from build123d import *

# Parameters (mm, degrees)
SKETCH_1_W             = 15
SKETCH_1_H             = 26
EXTRUDE_1_DEPTH        = 40
HOLE_WIZARD_M6_1_D     = 5
HOLE_WIZARD_M6_1_DEPTH = 15
HOLE_WIZARD_M6_1_TIP   = 1.502151548
HOLE_WIZARD_M6_2_D     = 5
HOLE_WIZARD_M6_2_DEPTH = 15
HOLE_WIZARD_M6_2_TIP   = 1.502151548
CHAMFER_2_SIZE         = 10


with BuildPart() as part:
    # 草图1 → 凸台-拉伸1 (new body)
    with BuildSketch(Plane.XY):
        Rectangle(SKETCH_1_W, SKETCH_1_H)
    extrude(amount=EXTRUDE_1_DEPTH)

    # M6 螺纹孔1
    with Locations(Plane(origin=(0, 13, 0), x_dir=(1, 0, 0), z_dir=(0, 1, 0))):
        with Locations((0, -12), (0, -28)):
            Hole(HOLE_WIZARD_M6_1_D / 2, depth=HOLE_WIZARD_M6_1_DEPTH)
            with Locations((0, 0, -(HOLE_WIZARD_M6_1_DEPTH + HOLE_WIZARD_M6_1_TIP / 2))):  # 118° drill point
                Cone(0, HOLE_WIZARD_M6_1_D / 2, HOLE_WIZARD_M6_1_TIP, mode=Mode.SUBTRACT)

    # M6 螺纹孔2
    with Locations(Plane(origin=(0, 0, 0), x_dir=(-1, 0, 0), z_dir=(0, 0, -1))):
        with Locations((0, 0)):
            Hole(HOLE_WIZARD_M6_2_D / 2, depth=HOLE_WIZARD_M6_2_DEPTH)
            with Locations((0, 0, -(HOLE_WIZARD_M6_2_DEPTH + HOLE_WIZARD_M6_2_TIP / 2))):  # 118° drill point
                Cone(0, HOLE_WIZARD_M6_2_D / 2, HOLE_WIZARD_M6_2_TIP, mode=Mode.SUBTRACT)

    # 倒角2
    chamfer_2_edges = [part.edges().sort_by_distance(p)[0] for p in [
        (0, -13, 40),
    ]]
    chamfer(chamfer_2_edges, length=CHAMFER_2_SIZE)


solid = part.part
The model under review builds one solid part; all positions refer to its coordinate system, in mm. A direction names the side the tool comes from. Round coordinates to 2 decimals unless told otherwise and drop trailing zeros. Loops run counter-clockwise (first coordinate to the right, second up) from the corner with the lowest first, then second, coordinate; pieces in that order, holes last. Notation, with made-up numbers: M 13.25,52 L 36.25,52 A32 ccw 36.25,87 Z; hole C 82.25,-37 d4. An arc over 180 degrees is marked long. Answer as a JSON object with one key per item and string values.
Item 1: We need section A-A, the plane y = 7. State the section outline as (x, z) points, and give its area (3 significant figures).
Check sheet entries:
{"outline": "M -7.5,0 L 7.5,0 L 7.5,40 L -7.5,40 Z; hole C 0,12 d5; hole C 0,28 d5", "area": "561 mm2"}
Item 2: For line 1 along Z through (x, y) = (0, 7); line 2 along X through (y, z) = (0, 13.2); line 3 along Y through (x, z) = (0, 14.25), list the stretches that pass through material, from the lowest coordinate up.
Check sheet entries:
{"line 1": "0 to 9.5, 14.5 to 25.5, 30.5 to 40", "line 2": "-7.5 to -2.5, 2.5 to 7.5", "line 3": "-13 to -2.5"}
Item 3: We need section B-B, the plane x = -6. State the section outline as (y, z) points.
Check sheet entries:
{"outline": "M -13,0 L 13,0 L 13,40 L -3,40 L -13,30 Z"}
Item 4: The part is to be moulded in two halves that separate along Z. For faces 1 (the face through (0, 3, 0)), 2 (the face through (0, 13, 20)), 3 (the face through (0.33, 5.4, 25.52)), say which applies: +Z half, -Z half, draft (parallel to the pull), parting line (faces both ways), or undercut.
Check sheet entries:
{"face 1": "-Z half", "face 2": "draft", "face 3": "undercut"}
Item 5: Tool access review of faces 4 (the face through (0, -13, 15)), 5 (the face through (-0.54, -2.44, 14.19)), 6 (the face through (2.5, -1.2, 12)): name each direction out of +Z, -Z, +X, -X, +Y, -Y from which nothing blocks a thin tool from reaching the whole face with its end or side.
Check sheet entries:
{"face 4": "+Z, -Z, +X, -X, -Y", "face 5": "-Z", "face 6": "+Y"}
Item 6: Clearance check with a flat-ended pin moving along its axis: P1, Ø4.5, axis at x = 0, y = 0, coming from the -Z side. State where the tip first meets the part, or that it passes through.
Check sheet entries:
{"P1": "z = 15.15"}
